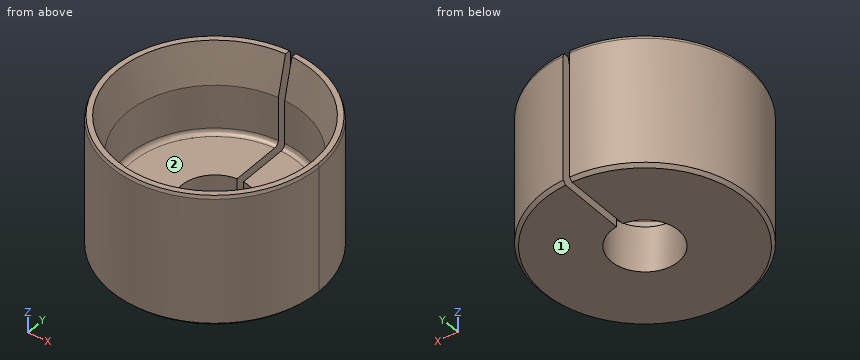
```python
from build123d import *

# Parameters (mm, degrees)
SKETCH_1_R          = 32.5
EXTRUDE_1_DEPTH     = 41.25
SKETCH_2_R          = 27.5
CUT_EXTRUDE_1_DEPTH = 27
HOLE_WIZARD_M24_1_D = 21
SKETCH_4_W          = 2
SKETCH_4_H          = 41.62847608
CUT_EXTRUDE_2_DEPTH = 62.758096635
CHAMFER_1_SIZE      = 1
CHAMFER_2_SIZE      = 1
CHAMFER_2_SIZE2     = 0.363970234
FILLET_1_R          = 1.5


with BuildPart() as part:
    # 草图1 → 凸台-拉伸1 (new body)
    with BuildSketch(Plane.XY):
        Circle(SKETCH_1_R)
    extrude(amount=EXTRUDE_1_DEPTH)

    # 草图2 → 切除-拉伸1 (cut)
    with BuildSketch(Plane.XY.offset(41.25)):
        Circle(SKETCH_2_R)
    extrude(amount=-CUT_EXTRUDE_1_DEPTH, mode=Mode.SUBTRACT)

    # M24 螺纹孔1 (through all)
    with Locations(Plane(origin=(0, 0, 0), x_dir=(-1, 0, 0), z_dir=(0, 0, -1))):
        with Locations((0, 0)):
            Hole(HOLE_WIZARD_M24_1_D / 2)

    # 草图4 → 切除-拉伸2 (cut, through all)
    with BuildSketch(Plane(origin=(0, 0, 0), x_dir=(-1, 0, 0), z_dir=(0, 0, -1))):
        with Locations((0, 16.25)):
            Rectangle(SKETCH_4_W, SKETCH_4_H)
    extrude(amount=-CUT_EXTRUDE_2_DEPTH, mode=Mode.SUBTRACT)

    # 草图5 → 切除-旋转1 (revolve, cut)
    with BuildSketch(Plane(origin=(0, 0, 0), x_dir=(0, 0, -1), z_dir=(1, 0, 0))):
        Polygon((-44.25, 27.481812167), (-29.25, 27.481812167), (-44.25, 31.22173221), align=None)
    revolve(axis=Axis((0, -0.007694129, 41.25), (0, 0.00018652434146350927, -0.9999999826043349)), mode=Mode.SUBTRACT)

    # 倒角1
    chamfer_1_edges = [part.edges().sort_by_distance(p)[0] for p in [
        (-22.624654693, -23.331845191, 0),
    ]]
    chamfer(chamfer_1_edges, length=CHAMFER_1_SIZE)

    # 倒角2
    chamfer_2_edges = [part.edges().sort_by_distance(p)[0] for p in [
        (-22.624654693, -23.331845191, 41.25),
    ]]
    chamfer_2_side = [part.faces().sort_by_distance(p)[0] for p in [
        (-22.624654693, -23.331845191, 21.125),
    ]]
    chamfer(chamfer_2_edges, length=CHAMFER_2_SIZE, length2=CHAMFER_2_SIZE2, reference=chamfer_2_side[0])

    # 圆角1
    fillet_1_edges = [part.edges().sort_by_distance(p)[0] for p in [
        (-19.088609169, -19.795832895, 14.25),
    ]]
    fillet(fillet_1_edges, radius=FILLET_1_R)


solid = part.part
```
Design review of the part built by this model. Coordinates are the model's own, in mm. Face numbers are marked on the shaded views. Coordinates: 2 decimals unless noted, no trailing zeros. Loops run counter-clockwise (first coordinate to the right, second up) from the corner with the lowest first, then second, coordinate; pieces in that order, holes last. Notation, with made-up numbers: (-27.5, 19.5) -> (4.5, 19.5) arc R17 ccw to (4.5, 45.5) -> close; hole circle Ø9 at (25, -9.75). An arc over 180 degrees is marked (long way). Answer as a JSON object with one key per item and string values.
Q1. Take a section at A-A on x = 0. Give the boundary of the cut face in (y, z), plus the area to 3 significant figures.
Answer block:
{"outline": "(-32.5, 1) -> (-31.5, 0) -> (-10.5, 0) -> (-10.5, 14.25) -> (-26, 14.25) arc R1.5 cw to (-27.5, 15.75) -> (-27.5, 29.27) -> (-30.49, 41.25) -> (-32.14, 41.25) -> (-32.5, 40.25) -> close", "area": "430 mm^2"}
Q2. To check wall thickness, follow L1, parallel to X at y = 0, z = 20.25; L2, parallel to X at y = 0, z = 9.5; L3, parallel to Y at x = 0, z = 6. State the ranges of each line that lie inside material, in increasing order.
Answer block:
{"L1": "x = -32.5 to -27.5, 27.5 to 32.5", "L2": "x = -32.5 to -10.5, 10.5 to 32.5", "L3": "y = -32.5 to -10.5"}
Q3. Clearance check with flat-ended pins moving along their axes: pin 1 Ø2 at (y, z) = (-25, 9.5) entering from +X; pin 2 Ø1 at (x, y) = (13, 1.5) entering from +Z; pin 3 Ø17.5 at (y, z) = (23.5, 21.5) entering from +X; pin 4 Ø5 at (x, y) = (-21, -6) entering from -Z. State where each tip first meets the part, or that it passes through.
Answer block:
{"pin 1": "stops at x = 21.91", "pin 2": "stops at z = 14.25", "pin 3": "stops at x = 28.96", "pin 4": "stops at z = 0"}
Q4. The part is to be moulded in two halves that separate along Y. For the marked faces 1 and 2, say which applies: +Y half, -Y half, draft (parallel to the pull), parting line (faces both ways), or undercut.
Answer block:
{"face 1": "draft", "face 2": "undercut"}
Q5. Take a section at B-B on z = 18.5. Give the boundary of the cut face in (x, y), plus the area to 3 significant figures.
Answer block:
{"outline": "(-1, 27.48) -> (-1, 32.48) arc R32.5 ccw (long way) to (1, 32.48) -> (1, 27.48) arc R27.5 cw (long way) to start", "area": "932 mm^2"}
Q6. Take a section at C-C on z = 7. Give the boundary of the cut face in (x, y), plus the area to 3 significant figures.
Answer block:
{"outline": "(-1, 10.45) -> (-1, 32.48) arc R32.5 ccw (long way) to (1, 32.48) -> (1, 10.45) arc R10.5 cw (long way) to start", "area": "2,930 mm^2"}
